```python
from build123d import *

# Parameters (mm, degrees)
BOSS_EXTRUDE1_DEPTH = 45
CUT_EXTRUDE1_REACH  = 72.774
SKETCH2_R           = 3.3
CUT_EXTRUDE2_REACH  = 74.201
SKETCH3_R           = 2.25
CUT_EXTRUDE3_REACH  = 74.201
FILLET1_R           = 5


with BuildPart() as part:
    # Sketch1 → Boss-Extrude1 (new body)
    with BuildSketch(Plane.XY):
        with BuildLine():
            Line((0, 0), (0, 17))
            ThreePointArc((0, 17), (1.464466094, 20.535533906), (5, 22))
            Line((5, 22), (52, 22))
            Line((52, 22), (52, 20))
            Line((52, 20), (5, 20))
            ThreePointArc((5, 20), (2.878679656, 19.121320344), (2, 17))
            Line((2, 17), (2, 0))
            Line((2, 0), (0, 0))
        make_face()
    extrude(amount=BOSS_EXTRUDE1_DEPTH)

    # Sketch2 → Cut-Extrude1 (cut, up to next)
    with BuildSketch(Plane(origin=(2, 0, 0), x_dir=(0, 0, -1), z_dir=(1, 0, 0)), mode=Mode.PRIVATE) as cut_extrude1_sk1:
        with Locations(Location((-37.5, 9, 0), (0, 0, 90))):
            Circle(SKETCH2_R)
    cut_extrude1_tool1 = extrude(cut_extrude1_sk1.sketch, amount=-CUT_EXTRUDE1_REACH, mode=Mode.PRIVATE) & part.part
    # Sketch2 → Cut-Extrude1 (cut, up to next)
    with BuildSketch(Plane(origin=(2, 0, 0), x_dir=(0, 0, -1), z_dir=(1, 0, 0)), mode=Mode.PRIVATE) as cut_extrude1_sk2:
        with Locations(Location((-7.5, 9, 0), (0, 0, 90))):
            Circle(SKETCH2_R)
    cut_extrude1_tool2 = extrude(cut_extrude1_sk2.sketch, amount=-CUT_EXTRUDE1_REACH, mode=Mode.PRIVATE) & part.part
    add(cut_extrude1_tool1.solids().sort_by_distance((2, 9, 37.5))[0], mode=Mode.SUBTRACT)
    add(cut_extrude1_tool2.solids().sort_by_distance((2, 9, 7.5))[0], mode=Mode.SUBTRACT)

    # Sketch3 → Cut-Extrude2 (cut, up to next)
    with BuildSketch(Plane(origin=(0, 22, 0), x_dir=(1, 0, 0), z_dir=(0, 1, 0)), mode=Mode.PRIVATE) as cut_extrude2_sk1:
        with Locations(Location((35, -22.5, 0), (0, 0, 270))):
            Circle(SKETCH3_R)
    cut_extrude2_tool1 = extrude(cut_extrude2_sk1.sketch, amount=-CUT_EXTRUDE2_REACH, mode=Mode.PRIVATE) & part.part
    # Sketch3 → Cut-Extrude2 (cut, up to next)
    with BuildSketch(Plane(origin=(0, 22, 0), x_dir=(1, 0, 0), z_dir=(0, 1, 0)), mode=Mode.PRIVATE) as cut_extrude2_sk2:
        with Locations(Location((47, -22.5, 0), (0, 0, 270))):
            Circle(SKETCH3_R)
    cut_extrude2_tool2 = extrude(cut_extrude2_sk2.sketch, amount=-CUT_EXTRUDE2_REACH, mode=Mode.PRIVATE) & part.part
    add(cut_extrude2_tool1.solids().sort_by_distance((35, 22, 22.5))[0], mode=Mode.SUBTRACT)
    add(cut_extrude2_tool2.solids().sort_by_distance((47, 22, 22.5))[0], mode=Mode.SUBTRACT)

    # Sketch4 → Cut-Extrude3 (cut, up to next)
    with BuildSketch(Plane(origin=(0, 22, 0), x_dir=(1, 0, 0), z_dir=(0, 1, 0)), mode=Mode.PRIVATE) as cut_extrude3_sk1:
        Polygon((5, 0), (52, -11), (52, 0), align=None)
    cut_extrude3_tool1 = extrude(cut_extrude3_sk1.sketch, amount=-CUT_EXTRUDE3_REACH, mode=Mode.PRIVATE) & part.part
    # Sketch4 → Cut-Extrude3 (cut, up to next)
    with BuildSketch(Plane(origin=(0, 22, 0), x_dir=(1, 0, 0), z_dir=(0, 1, 0)), mode=Mode.PRIVATE) as cut_extrude3_sk2:
        Polygon((5, -45), (52, -34), (52, -45), align=None)
    cut_extrude3_tool2 = extrude(cut_extrude3_sk2.sketch, amount=-CUT_EXTRUDE3_REACH, mode=Mode.PRIVATE) & part.part
    add(cut_extrude3_tool1.solids().sort_by_distance((36.333333, 22, 3.666667))[0], mode=Mode.SUBTRACT)
    add(cut_extrude3_tool2.solids().sort_by_distance((36.333333, 22, 41.333333))[0], mode=Mode.SUBTRACT)

    # Fillet1
    fillet1_edges = [part.edges().sort_by_distance(p)[0] for p in [
        (1, 0, 0),
        (1, 0, 45),
        (52, 21, 11),
        (52, 21, 34),
    ]]
    fillet(fillet1_edges, radius=FILLET1_R)


solid = part.part
```
Work out the finished part from the listing and answer in its coordinate system (mm). A direction names the side the tool comes from. Give positions to 0.01 mm unless a question says otherwise; leave off trailing zeros. Loops run counter-clockwise (first coordinate to the right, second up) from the corner with the lowest first, then second, coordinate; pieces in that order, holes last. Notation, with made-up numbers: (-0.75, -8.75) -> (38.25, -8.75) arc R28 ccw to (38.25, 27.25) -> close; hole circle Ø8 at (-27.75, 19.5). An arc over 180 degrees is marked (long way). One line per question, with ' | ' between items. Start each with the question number.
1) Straight lines are drawn through the part: L1, parallel to Z at x = 1, y = 9; L2, parallel to X at y = 20.9, z = 22.5; L3, parallel to Y at x = 15, z = 10. For each, find the intervals that lie inside material, in ascending order.
2) Determine the mould class of faces 1 (the face through (26.27, 21.01, 4.98)), 2 (the face through (0, 8, 22)), 3 (the face through (36.897, 21.014, 23.71)) for opening direction X: +X half, -X half, draft (parallel to the pull), parting line (faces both ways), or undercut.
3) Section B-B, the plane y = 9 is taken. Determine the outline of the cut face in (x, z).
4) Section A-A, the plane z = 22.5 is taken. Determine the outline of the cut face in (x, y).
5) Section D-D, the plane z = 7.5 is taken. Determine the outline of the cut face in (x, y), then the cut area to 3 significant figures.
6) Section C-C, the plane x = 47 is taken. Determine the outline of the cut face in (y, z).
7) Each of these flat-tipped pins is pushed along its axis until it touches: pin 1 (6 mm diameter, centred on x = 21.5, y = 17.5, fed in from +Z); pin 2 (8 mm diameter, centred on x = 32, z = 35.5, fed in from -Y); pin 3 (6 mm diameter, centred on x = 19, y = 18.5, fed in from +Z). Where does it stop, or does it pass through?
8) For faces 4 (the face through (2, 9, 22)), 5 (the face through (52, 21, 22)), determine the directions among +Z, -Z, +X, -X, +Y, -Y from which every point of the face is accessible in a straight line to the end or side of a thin tool.
Resolved:
1) L1: 0 to 4.2, 10.8 to 34.2, 40.8 to 45 | L2: 1.87 to 32.75, 37.25 to 44.75, 49.25 to 52 | L3: 20 to 22
2) face 1: +X half | face 2: -X half | face 3: undercut
3) outline: (0, 0) -> (2, 0) -> (2, 4.2) -> (0, 4.2) -> close; (0, 10.8) -> (2, 10.8) -> (2, 34.2) -> (0, 34.2) -> close; (0, 40.8) -> (2, 40.8) -> (2, 45) -> (0, 45) -> close
4) outline: (0, 0) -> (2, 0) -> (2, 17) arc R3 cw to (5, 20) -> (32.75, 20) -> (32.75, 22) -> (5, 22) arc R5 ccw to (0, 17) -> close; (37.25, 20) -> (44.75, 20) -> (44.75, 22) -> (37.25, 22) -> close; (49.25, 20) -> (52, 20) -> (52, 22) -> (49.25, 22) -> close
5) outline: (0, 0) -> (2, 0) -> (2, 5.7) -> (0, 5.7) -> close; (0, 12.3) -> (2, 12.3) -> (2, 17) arc R3 cw to (5, 20) -> (37.05, 20) -> (37.05, 22) -> (5, 22) arc R5 ccw to (0, 17) -> close | area: 97.5 mm2
6) outline: (20, 9.83) -> (22, 9.83) -> (22, 20.25) -> (20, 20.25) -> close; (20, 24.75) -> (22, 24.75) -> (22, 35.17) -> (20, 35.17) -> close
7) pin 1: z = 41.53 | pin 2: y = 20 | pin 3: z = 42.33
8) face 4: +Z, -Z, +X, -Y | face 5: +Z, -Z, +X, +Y, -Y
